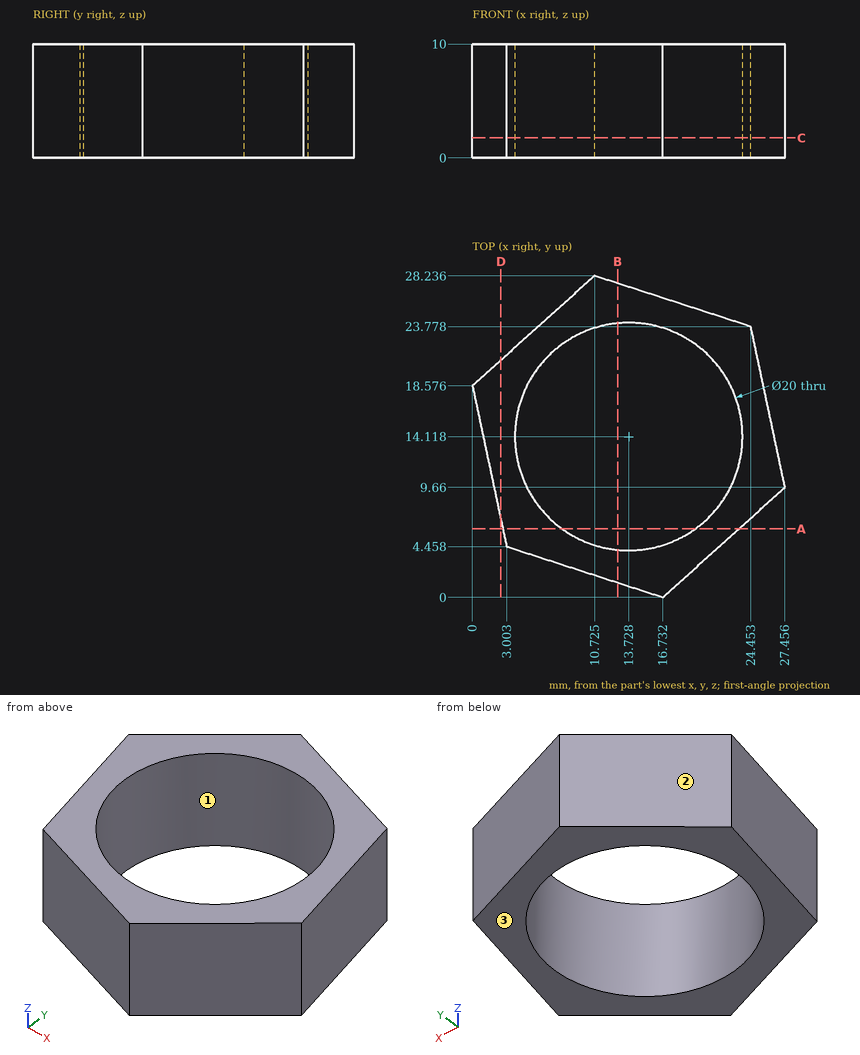
Geometry check sheet. Reference: drawing and pictorial views, mm from the part's lowest x, y, z. Give positions to 0.01 mm unless a question says otherwise; leave off trailing zeros. Loops run counter-clockwise (first coordinate to the right, second up) from the corner with the lowest first, then second, coordinate; pieces in that order, holes last. Notation, with made-up numbers: (20.25, 71) -> (27.25, 71) arc R29 ccw to (27.25, 104) -> close; hole circle Ø2 at (28, 74). An arc over 180 degrees is marked (long way). Answer in a Markdown table with one row per item. Add a question column.
1) Cross-section at A-A on y = 6. Record the boundary of the cut face in (x, z) (1 decimal).
2) Material ranges on probe 1 along X at (y, z) = (10.75, 3.5) (1 decimal); probe 2 along X at (y, z) = (9.5, 5.25) (1 decimal); probe 3 along Y at (x, z) = (18.25, 1.25) (1 decimal), recorded low to high. Write a range as from..to.
3) Draft check along X on the marked faces 1, 2 and 3. Enter one of: pulls with the +X half, pulls with the -X half, needs draft (parallel to the pull), parting line crosses it, or undercut.
4) Cross-section at C-C on z = 1.75. Record the boundary of the cut face in (x, y) (1 decimal).
5) Cross-section at D-D on x = 2.5. Record the boundary of the cut face in (y, z) (1 decimal), and give its area (3 significant figures).
6) Cross-section at B-B on x = 12.75. Record the boundary of the cut face in (y, z) (1 decimal).
7) Gauge pin test, flat ends, axial feed: P1, Ø6, axis at y = 5, z = 5.5, coming from the +X side (1 decimal); P2, Ø4, axis at y = 8, z = 6, coming from the -X side (1 decimal); P3, Ø3, axis at x = 6, y = 16, coming from the -Z side; P4, Ø1.5, axis at x = 18.5, z = 5, coming from the -Y side. Record the tip position at first contact, or that the pin passes through.
Outcome:
| question | item | result |
|---|---|---|
| 1 | outline | (2.7, 0) -> (7.9, 0) -> (7.9, 10) -> (2.7, 10) -> close; (19.6, 0) -> (23.4, 0) -> (23.4, 10) -> (19.6, 10) -> close |
| 2 | probe 1 | x = 1.7..4.3, 23.1..27.2 |
| 2 | probe 2 | x = 1.9..4.9, 22.6..27.3 |
| 2 | probe 3 | y = 1.4..5.2, 23..25.8 |
| 3 | face 1 | undercut |
| 3 | face 2 | pulls with the -X half |
| 3 | face 3 | needs draft |
| 4 | outline | (0, 18.6) -> (3, 4.5) -> (16.7, 0) -> (27.5, 9.7) -> (24.5, 23.8) -> (10.7, 28.2) -> close; hole circle Ø20 at (13.7, 14.1) |
| 5 | outline | (6.8, 0) -> (20.8, 0) -> (20.8, 10) -> (6.8, 10) -> close |
| 5 | area | 140 mm^2 |
| 6 | outline | (1.3, 0) -> (4.2, 0) -> (4.2, 10) -> (1.3, 10) -> close; (24.1, 0) -> (27.6, 0) -> (27.6, 10) -> (24.1, 10) -> close |
| 7 | P1 | stops at x = 25.6 |
| 7 | P2 | stops at x = 1.8 |
| 7 | P3 | passes through |
| 7 | P4 | stops at y = 0.92 |
